```python
from build123d import *

# Parameters (mm, degrees)
SKETCH1_W               = 126
SKETCH1_H               = 150
BOSS_EXTRUDE1_DEPTH     = 6.5
SKETCH2_R               = 1.5
CUT_EXTRUDE1_DEPTH      = 10
MIRROR2_COPY_1_SKETCH_R = 1.5
MIRROR2_COPY_1_DEPTH    = 10
FILLET1_R               = 10


with BuildPart() as part:
    # Sketch1 → Boss-Extrude1 (new body)
    with BuildSketch(Plane(origin=(0, 0, 0), x_dir=(1, 0, 0), z_dir=(0, 1, 0))):
        Rectangle(SKETCH1_W, SKETCH1_H)
    extrude(amount=BOSS_EXTRUDE1_DEPTH)

    # Sketch2 → Cut-Extrude1 (cut)
    with BuildSketch(Plane(origin=(0, 6.5, 0), x_dir=(1, 0, 0), z_dir=(0, 1, 0))):
        with Locations(Location((-55.5, 33, 0), (0, 0, 270))):
            Circle(SKETCH2_R)
        with Locations(Location((-48, 33, 0), (0, 0, 90))):
            Circle(SKETCH2_R)
        with Locations(Location((-48, 53, 0), (0, 0, 270))):
            Circle(SKETCH2_R)
        with Locations(Location((-55.5, 53, 0), (0, 0, 90))):
            Circle(SKETCH2_R)
    cut_extrude1 = extrude(amount=-CUT_EXTRUDE1_DEPTH, mode=Mode.SUBTRACT)

    # Mirror1: Cut-Extrude1 across plane
    add(cut_extrude1.mirror(Plane(origin=(0, 0, 0), x_dir=(0, 0, 1), z_dir=(1, 0, 0))), mode=Mode.SUBTRACT)

    # Mirror2: Cut-Extrude1 across plane
    add(cut_extrude1.mirror(Plane.XY), mode=Mode.SUBTRACT)

    # Mirror2 copy 1 sketch → Mirror2 copy 1 (cut)
    with BuildSketch(Plane(origin=(0, 6.5, 0), x_dir=(-1, 0, 0), z_dir=(0, 1, 0))):
        with Locations(Location((-55.5, 33, 0), (0, 0, 270))):
            Circle(MIRROR2_COPY_1_SKETCH_R)
        with Locations(Location((-48, 33, 0), (0, 0, 90))):
            Circle(MIRROR2_COPY_1_SKETCH_R)
        with Locations(Location((-48, 53, 0), (0, 0, 270))):
            Circle(MIRROR2_COPY_1_SKETCH_R)
        with Locations(Location((-55.5, 53, 0), (0, 0, 90))):
            Circle(MIRROR2_COPY_1_SKETCH_R)
    extrude(amount=-MIRROR2_COPY_1_DEPTH, mode=Mode.SUBTRACT)

    # Fillet1
    fillet1_edges = [part.edges().sort_by_distance(p)[0] for p in [
        (63, 3.25, 75),
        (-63, 3.25, 75),
        (-63, 3.25, -75),
        (63, 3.25, -75),
    ]]
    fillet(fillet1_edges, radius=FILLET1_R)


solid = part.part
```
Source: CAD feature listing. Evaluate the final solid. Frame: model axes, mm. Give positions to 0.01 mm unless a question says otherwise; leave off trailing zeros.
1. Pull-direction query (Z, two-part tool) for faces 1 (the face through (49.464, 3.296, 53.325)), 2 (the face through (-1, 3, -75)), 3 (the face through (-1, 6.5, -1)); classes: +Z half, -Z half, draft (parallel to the pull), parting line (faces both ways), or undercut.
2. Material intervals for line 1 along X through (y, z) = (1.5, 53); line 2 along Z through (x, y) = (-56.5, 3.5), sorted ascending.
3. First-contact query: pin 1 (5 mm diameter, centred on x = 55.5, z = 33, fed in from -Y); pin 2 (2.5 mm diameter, centred on x = -55.5, z = 33, fed in from -Y). Flat tips, straight axial feed; report the tip coordinate or a pass-through.
Output values:
1. face 1: undercut
1. face 2: -Z half
1. face 3: draft
2. line 1: x = -63 to -57, -54 to -49.5, -46.5 to 46.5, 49.5 to 54, 57 to 63
2. line 2: z = -74.37 to -54.12, -51.88 to -34.12, -31.88 to 31.88, 34.12 to 51.88, 54.12 to 74.37
3. pin 1: stops at y = 0
3. pin 2: passes through
